```python
from build123d import *

# Parameters (mm, degrees)
SKETCH_1_W                = 82
SKETCH_1_H                = 137
EXTRUDE_1_DEPTH           = 10
SKETCH_4_R                = 10.5
CUT_EXTRUDE_3_DEPTH       = 81.456509991
FILLET_9_R                = 10
HOLE_WIZARD_2_D           = 4.3
HOLE_WIZARD_2_CBORE_D     = 8
HOLE_WIZARD_2_CBORE_DEPTH = 4.6
HOLE_WIZARD_M4_2_D        = 3.3
HOLE_WIZARD_M4_2_DEPTH    = 18.5
HOLE_WIZARD_M4_2_TIP      = 0.991420021
MM_2_D                    = 21.1
HOLE_WIZARD_M4_3_D        = 3.3
MM_2_2_D                  = 5
MM_2_2_DEPTH              = 10.1
MM_2_2_TIP                = 1.502151548
HOLE_WIZARD_M6_1_D        = 5
HOLE_WIZARD_M6_1_DEPTH    = 15
HOLE_WIZARD_M6_1_TIP      = 1.502151548
HOLE_WIZARD_M6_4_D        = 5


with BuildPart() as part:
    # 草图1 → 凸台-拉伸1 (new body)
    with BuildSketch(Plane(origin=(0, 0, 0), x_dir=(1, 0, 0), z_dir=(0, 1, 0))):
        Rectangle(SKETCH_1_W, SKETCH_1_H)
    extrude(amount=EXTRUDE_1_DEPTH)

    # 草图4 → 切除-拉伸3 (cut, through all)
    with BuildSketch(Plane(origin=(0, 10, 0), x_dir=(1, 0, 0), z_dir=(0, 1, 0))):
        with Locations(Location((0, -55, 0), (0, 0, 270))):
            Circle(SKETCH_4_R)
    extrude(amount=-CUT_EXTRUDE_3_DEPTH, mode=Mode.SUBTRACT)

    # 圆角9
    fillet_9_edges = [part.edges().sort_by_distance(p)[0] for p in [
        (41, 5, 68.5),
        (-41, 5, 68.5),
    ]]
    fillet(fillet_9_edges, radius=FILLET_9_R)

    # 打孔尺寸(%根据)开槽圆柱头螺钉的类型2 (through all)
    with Locations(Plane(origin=(0, 10, 0), x_dir=(1, 0, 0), z_dir=(0, 1, 0))):
        with Locations((-16.5, -55), (16.5, -55)):
            CounterBoreHole(HOLE_WIZARD_2_D / 2, HOLE_WIZARD_2_CBORE_D / 2, HOLE_WIZARD_2_CBORE_DEPTH)

    # M4 螺纹孔2
    with Locations(Plane(origin=(0, 0, -68.5), x_dir=(-1, 0, 0), z_dir=(0, 0, -1))):
        with Locations((-15, 5), (15, 5)):
            Hole(HOLE_WIZARD_M4_2_D / 2, depth=HOLE_WIZARD_M4_2_DEPTH)
            with Locations((0, 0, -(HOLE_WIZARD_M4_2_DEPTH + HOLE_WIZARD_M4_2_TIP / 2))):  # 118° drill point
                Cone(0, HOLE_WIZARD_M4_2_D / 2, HOLE_WIZARD_M4_2_TIP, mode=Mode.SUBTRACT)

    # mm _2 (through all)
    with Locations(Plane(origin=(0, 10, 0), x_dir=(1, 0, 0), z_dir=(0, 1, 0))):
        with Locations((-25, -14.5), (25, -14.5)):
            Hole(MM_2_D / 2)

    # M4 螺纹孔3 (through all)
    with Locations(Plane(origin=(0, 0, 0), x_dir=(-1, 0, 0), z_dir=(0, -1, 0))):
        with Locations((-13.686291501, -3.186291501), (-36.313708499, -3.186291501), (-36.313708499, -25.813708499), (-13.686291501, -25.813708499)):
            hole_wizard_m4_3 = Hole(HOLE_WIZARD_M4_3_D / 2)

    # 镜向2: M4 螺纹孔3 across plane
    add(hole_wizard_m4_3.mirror(Plane(origin=(0, 0, 0), x_dir=(0, 0, 1), z_dir=(1, 0, 0))), mode=Mode.SUBTRACT)

    # mm _2 2
    with Locations(Plane(origin=(0, 0, -68.5), x_dir=(-1, 0, 0), z_dir=(0, 0, -1))):
        with Locations((32.5, 5), (-32.5, 5)):
            Hole(MM_2_2_D / 2, depth=MM_2_2_DEPTH)
            with Locations((0, 0, -(MM_2_2_DEPTH + MM_2_2_TIP / 2))):  # 118° drill point
                Cone(0, MM_2_2_D / 2, MM_2_2_TIP, mode=Mode.SUBTRACT)

    # M6 螺纹孔1
    with Locations(Plane(origin=(0, 10, 0), x_dir=(1, 0, 0), z_dir=(0, 1, 0))):
        with Locations((0, 49.5)):
            Hole(HOLE_WIZARD_M6_1_D / 2, depth=HOLE_WIZARD_M6_1_DEPTH)
            with Locations((0, 0, -(HOLE_WIZARD_M6_1_DEPTH + HOLE_WIZARD_M6_1_TIP / 2))):  # 118° drill point
                Cone(0, HOLE_WIZARD_M6_1_D / 2, HOLE_WIZARD_M6_1_TIP, mode=Mode.SUBTRACT)

    # M6 螺纹孔4 (through all)
    with Locations(Plane(origin=(0, 10, 0), x_dir=(1, 0, 0), z_dir=(0, 1, 0))):
        with Locations((0, 23.5)):
            Hole(HOLE_WIZARD_M6_4_D / 2)


solid = part.part
```
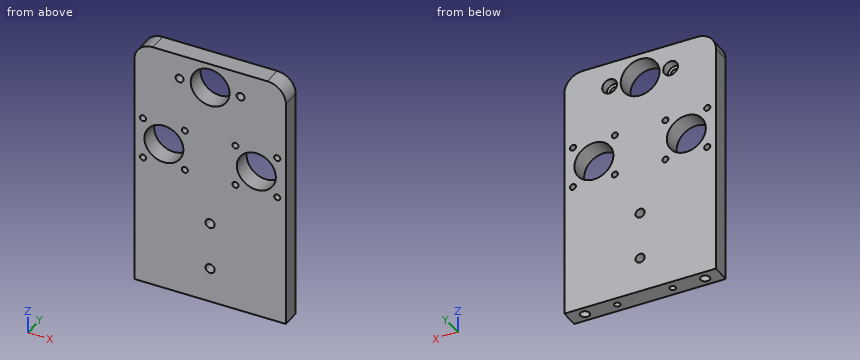
Model file for the job. Use its own axes, mm. Give positions to 0.01 mm unless a question says otherwise; leave off trailing zeros. Loops run counter-clockwise (first coordinate to the right, second up) from the corner with the lowest first, then second, coordinate; pieces in that order, holes last. Notation, with made-up numbers: (-3.5, 32) - (0.5, 32) arc R21 ccw to (0.5, 61) - close; hole circle Ø1 at (50, 84.5). An arc over 180 degrees is marked (long way). One line per item, written item: value. Start each with the question number.
1. Slice it at D-D (x = 27). List the corners of the cut face in (y, z).
2. Pin check, flat tips, straight feed: pin 1 (5 mm diameter, centred on x = 16.5, z = 55, fed in from +Y); pin 2 (2.5 mm diameter, centred on x = -15, y = 5, fed in from -Z). Stop position of each tip, or through.
3. Slice it at B-B (x = 0). List the corners of the cut face in (y, z).
4. Probe L1, parallel to X at y = 5, z = -62.75; L2, parallel to X at y = 2, z = 8.5; L3, parallel to X at y = 9.5, z = 57. List the from-to ranges inside material, lowest first. Write a range as from..to.
5. Slice it at A-A (z = 55). List the corners of the cut face in (x, y).
6. Slice it at C-C (z = 14.5). List the corners of the cut face in (x, y).
Solution:
1. outline: (0, -68.5) - (10, -68.5) - (10, 4.14) - (0, 4.14) - close; (0, 24.86) - (10, 24.86) - (10, 68.5) - (0, 68.5) - close
2. pin 1: stops at y = 5.4
2. pin 2: stops at z = -49.76
3. outline: (0, -68.5) - (10, -68.5) - (10, -52) - (0, -52) - close; (0, -47) - (10, -47) - (10, -26) - (0, -26) - close; (0, -21) - (10, -21) - (10, 44.5) - (0, 44.5) - close; (0, 65.5) - (10, 65.5) - (10, 68.5) - (0, 68.5) - close
4. L1: x = -41..-35, -30..-16.65, -13.35..13.35, 16.65..30, 35..41
4. L2: x = -41..-33.68, -16.32..16.32, 33.68..41
4. L3: x = -41..-19.96, -13.04..-10.31, 10.31..13.04, 19.96..41
5. outline: (-41, 0) - (-18.65, 0) - (-18.65, 5.4) - (-20.5, 5.4) - (-20.5, 10) - (-41, 10) - close; (-14.35, 0) - (-10.5, 0) - (-10.5, 10) - (-12.5, 10) - (-12.5, 5.4) - (-14.35, 5.4) - close; (10.5, 0) - (14.35, 0) - (14.35, 5.4) - (12.5, 5.4) - (12.5, 10) - (10.5, 10) - close; (18.65, 0) - (41, 0) - (41, 10) - (20.5, 10) - (20.5, 5.4) - (18.65, 5.4) - close
6. outline: (-41, 0) - (-35.55, 0) - (-35.55, 10) - (-41, 10) - close; (-14.45, 0) - (14.45, 0) - (14.45, 10) - (-14.45, 10) - close; (35.55, 0) - (41, 0) - (41, 10) - (35.55, 10) - close
